Check sheet for the drawn part. Datum: minimum x, y, z corner. Units: mm. Round coordinates to 2 decimals unless told otherwise and drop trailing zeros. Loops run counter-clockwise (first coordinate to the right, second up) from the corner with the lowest first, then second, coordinate; pieces in that order, holes last.
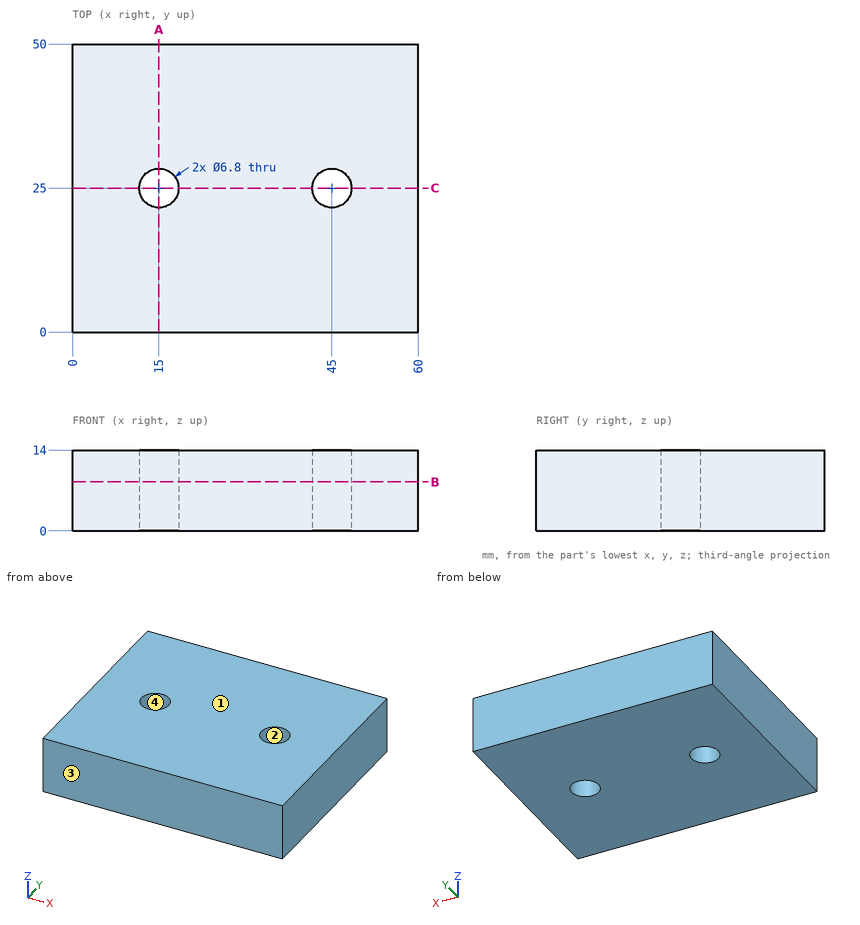
1) Scan lines: line 1 along Y through (x, z) = (15, 11); line 2 along Y through (x, z) = (48, 7.25). Record each from-to range of solid material in increasing order.
Report:
line 1: y = 0 to 21.6, 28.4 to 50
line 2: y = 0 to 23.4, 26.6 to 50
2) Sectioned sample at A-A, the plane x = 15. Record the cut outline in (y, z), then the cut area to 3 significant figures.
Report:
outline: (0, 0) - (21.6, 0) - (21.6, 14) - (0, 14) - close; (28.4, 0) - (50, 0) - (50, 14) - (28.4, 14) - close
area: 605 mm2
3) Sectioned sample at B-B, the plane z = 8.5. Record the cut outline in (x, y).
Report:
outline: (0, 0) - (60, 0) - (60, 50) - (0, 50) - close; hole circle Ø6.8 at (15, 25); hole circle Ø6.8 at (45, 25)
4) Mould release check, pull along Y, two halves, no side actions. Record for the marked faces 1, 2, 3 and 4: +Y half, -Y half, draft (parallel to the pull), parting line (faces both ways), or undercut.
Report:
face 1: draft
face 2: undercut
face 3: -Y half
face 4: undercut
5) Sectioned sample at C-C, the plane y = 25. Record the cut outline in (x, z), then the cut area to 3 significant figures.
Report:
outline: (0, 0) - (11.6, 0) - (11.6, 14) - (0, 14) - close; (18.4, 0) - (41.6, 0) - (41.6, 14) - (18.4, 14) - close; (48.4, 0) - (60, 0) - (60, 14) - (48.4, 14) - close
area: 650 mm2
